Here's how the part is built. I have some questions about the finished solid (model axes, mm). Face numbers are marked on the shaded views. Coordinates: 2 decimals unless noted, no trailing zeros. Write each loop counter-clockwise with the first axis right and the second up, starting at its lowest first coordinate (ties: lowest second). Pieces come first, ordered by that corner, then holes. Notation, with made-up numbers: (88, 37) -> (143, 37) arc R36 cw to (143, 75) -> close; hole circle Ø8 at (2, 72). An arc over 180 degrees is marked (long way). Put each result on its own line as item: value. Start each with the question number.
Item 1: I want a section at A-A, the plane x = 0. List the corners of the cut face in (y, z) for me.
Item 2: I want a section at C-C, the plane z = 13.75. List the corners of the cut face in (x, y) for me, then the cut area to 3 significant figures.
Item 3: If we mould it in two halves opening along X, with no side actions, what happens to the marked faces 1, 2 and 3? For each: released by +X, released by -X, zero draft, split by the parting line, or undercut.
Item 4: For pin 1 (7 mm diameter, centred on x = 3, y = 0, fed in from +Z); pin 2 (3 mm diameter, centred on x = -4, y = 4.5, fed in from +Z); pin 3 (12 mm diameter, centred on x = -7.5, z = 6.5, fed in from +Y); pin 4 (11 mm diameter, centred on x = 0, y = 0, fed in from +Z), each with a flat end and sliding along its axis, tell me the tip position at first contact or that it passes through.
Item 5: I need wall thicknesses on line 1 (Y direction, x = 0, z = 15); line 2 (Z direction, x = -5, y = 10.75); line 3 (X direction, y = -5, z = 4.75). Which ranges of each line are inside material? Lowest first, please. Write a range as [from, to].
Item 6: I want a section at D-D, the plane y = -9. List the corners of the cut face in (x, z) for me, then the cut area to 3 significant figures.
from build123d import *

# Parameters (mm, degrees)
SKETCH1_R           = 12
BOSS_EXTRUDE1_DEPTH = 3
SKETCH2_R           = 10
BOSS_EXTRUDE2_DEPTH = 18
SKETCH3_R           = 6
CUT_EXTRUDE1_DEPTH  = 26
CHAMFER1_SIZE       = 2


with BuildPart() as part:
    # Sketch1 → Boss-Extrude1 (new body)
    with BuildSketch(Plane.XY):
        Circle(SKETCH1_R)
    extrude(amount=BOSS_EXTRUDE1_DEPTH)

    # Sketch2 → Boss-Extrude2 (add)
    with BuildSketch(Plane.XY.offset(3)):
        Circle(SKETCH2_R)
    extrude(amount=BOSS_EXTRUDE2_DEPTH)

    # Sketch3 → Cut-Extrude1 (cut)
    with BuildSketch(Plane.XY.offset(21)):
        Circle(SKETCH3_R)
    extrude(amount=-CUT_EXTRUDE1_DEPTH, mode=Mode.SUBTRACT)

    # Chamfer1
    chamfer1_edges = [part.edges().sort_by_distance(p)[0] for p in [
        (-6, 0, 21),
    ]]
    chamfer(chamfer1_edges, length=CHAMFER1_SIZE)


solid = part.part
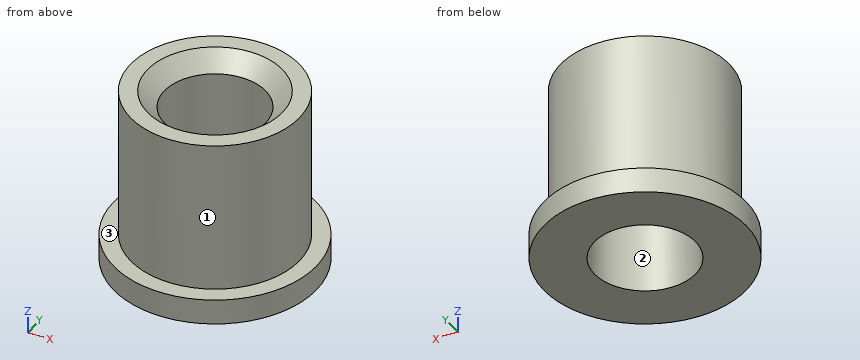
Calculated:
1. outline: (-12, 0) -> (-6, 0) -> (-6, 19) -> (-8, 21) -> (-10, 21) -> (-10, 3) -> (-12, 3) -> close; (6, 0) -> (12, 0) -> (12, 3) -> (10, 3) -> (10, 21) -> (8, 21) -> (6, 19) -> close
2. outline: circle Ø20 at (0, 0); hole circle Ø12 at (0, 0)
2. area: 201 mm2
3. face 1: split by the parting line
3. face 2: undercut
3. face 3: zero draft
4. pin 1: stops at z = 19.5
4. pin 2: stops at z = 20.52
4. pin 3: stops at y = 11.71
4. pin 4: passes through
5. line 1: y = [-10, -6], [6, 10]
5. line 2: z = [0, 3]
5. line 3: x = [-8.66, -3.32], [3.32, 8.66]
6. outline: (-7.94, 0) -> (7.94, 0) -> (7.94, 3) -> (4.36, 3) -> (4.36, 21) -> (-4.36, 21) -> (-4.36, 3) -> (-7.94, 3) -> close
6. area: 205 mm2
